from build123d import *

# Parameters (mm, degrees)
SKETCH_1_R          = 19
EXTRUDE_1_DEPTH     = 7
EXTRUDE_2_DEPTH     = 15
SKETCH_3_R          = 17.5
CUT_EXTRUDE_1_DEPTH = 2
SKETCH_4_R          = 15
CUT_EXTRUDE_2_DEPTH = 41.426888742
CHAMFER_1_SIZE      = 1


with BuildPart() as part:
    # 草图1 → 凸台-拉伸1 (new body)
    with BuildSketch(Plane.XY):
        Circle(SKETCH_1_R)
    extrude(amount=-EXTRUDE_1_DEPTH)

    # 草图2 → 凸台-拉伸2 (add)
    with BuildSketch(Plane(origin=(0, 0, -7), x_dir=(-1, 0, 0), z_dir=(0, 0, -1))):
        Polygon((13.279056191, -23), (26.558112383, 0), (13.279056191, 23), (-13.279056191, 23), (-26.558112383, 0), (-13.279056191, -23), align=None)
    extrude(amount=EXTRUDE_2_DEPTH)

    # 草图3 → 切除-拉伸1 (cut)
    with BuildSketch(Plane.XY):
        with Locations((-0.437352874, 0)):
            Circle(SKETCH_3_R)
    extrude(amount=-CUT_EXTRUDE_1_DEPTH, mode=Mode.SUBTRACT)

    # 草图4 → 切除-拉伸2 (cut, through all)
    with BuildSketch(Plane.XY.offset(-2)):
        Circle(SKETCH_4_R)
    extrude(amount=-CUT_EXTRUDE_2_DEPTH, mode=Mode.SUBTRACT)

    # 倒角1
    chamfer_1_edges = [part.edges().sort_by_distance(p)[0] for p in [
        (-15, 0, -22),
        (-15, 0, -2),
    ]]
    chamfer(chamfer_1_edges, length=CHAMFER_1_SIZE)


solid = part.part
Input: part model. Units: mm. Frame: model coordinates. A direction names the side the tool comes from. Give positions to 0.01 mm unless a question says otherwise; leave off trailing zeros. Loops run counter-clockwise (first coordinate to the right, second up) from the corner with the lowest first, then second, coordinate; pieces in that order, holes last. Notation, with made-up numbers: M 75,30.25 L 98,30.25 A3 cw 98,35.25 Z; hole C 69,-17 d10. An arc over 180 degrees is marked long. Use CSV: the item, a comma, the result in double quotes.
(1) Material intervals for L1, parallel to Y at x = 0, z = -15.25; L2, parallel to Z at x = -15.5, y = 15; L3, parallel to X at y = -1.5, z = -17.75, sorted ascending. Write a range as [from, to].
Outcome:
L1,"y = [-23, -15], [15, 23]"
L2,"z = [-22, -7]"
L3,"x = [-25.69, -14.92], [14.92, 25.69]"
(2) Section A-A, the plane z = -9.5. Return loops of the section in (x, y).
Outcome:
outline,"M -26.56,0 L -13.28,-23 L 13.28,-23 L 26.56,0 L 13.28,23 L -13.28,23 Z; hole C 0,0 d30"
(3) Pull-direction query (X, two-part tool) for faces 1 (the face through (-20.01, 11.34, -14.4)), 2 (the face through (-14.325, -10.648, -0.986)), 3 (the face through (20.01, -11.34, -14.4)); classes: pulls with the +X half, pulls with the -X half, needs draft (parallel to the pull), parting line crosses it, or undercut.
Outcome:
face 1,"pulls with the -X half"
face 2,"undercut"
face 3,"pulls with the +X half"
(4) Pin query (flat end, axial travel): P1, Ø10, axis at y = 8.5, z = -3.5, coming from the -X side; P2, Ø1, axis at y = 15.5, z = -10.5, coming from the -X side; P3, Ø5, axis at x = -2, y = 10, coming from the +Z side; P4, Ø4, axis at y = -1, z = -11, coming from the -X side. Return the tip coordinate at first contact, or that it passes through.
Outcome:
P1,"stops at x = -23.71"
P2,"stops at x = -17.9"
P3,"passes through"
P4,"stops at x = -26.56"
(5) Set-up query: faces 4 (the face through (0, -23, -14)), 5 (the face through (-4, -19, -7)). Return all of +Z, -Z, +X, -X, +Y, -Y with unobstructed straight access to the full face (end or side cutting, diameter ignored); none if empty.
Outcome:
face 4,"+Z, -Z, +X, -X, -Y"
face 5,"+Z"
(6) Section B-B, the plane x = 0. Return loops of the section in (y, z).
Outcome:
outline,"M -23,-22 L -16,-22 L -15,-21 L -15,-3 L -16,-2 L -17.49,-2 L -17.49,0 L -19,0 L -19,-7 L -23,-7 Z; M 15,-21 L 16,-22 L 23,-22 L 23,-7 L 19,-7 L 19,0 L 17.49,0 L 17.49,-2 L 16,-2 L 15,-3 Z"
(7) Section D-D, the plane x = 20.5. Return loops of the section in (y, z).
Outcome:
outline,"M -10.49,-22 L 10.49,-22 L 10.49,-7 L -10.49,-7 Z"
(8) Section C-C, the plane z = -4.5. Return loops of the section in (x, y), plus the area to 3 significant figures.
Outcome:
outline,"C 0,0 d38; hole C 0,0 d30"
area,"427 mm²"
